Read the model definition and answer for the solid it produces. Units are mm, in the model's axes. Give positions to 0.01 mm unless a question says otherwise; leave off trailing zeros. Write each loop counter-clockwise with the first axis right and the second up, starting at its lowest first coordinate (ties: lowest second). Pieces come first, ordered by that corner, then holes. Notation, with made-up numbers: (-6, 25) -> (43, 25) arc R18 cw to (43, 37) -> close; hole circle Ø10 at (14, 70). An arc over 180 degrees is marked (long way). Use a Markdown table: item, result.
from build123d import *

# Parameters (mm, degrees)
SKETCH_1_R      = 1.65
EXTRUDE_1_DEPTH = 1.6


with BuildPart() as part:
    # 草图1 → 凸台-拉伸1 (new, symmetric)
    with BuildSketch(Plane.XY):
        Polygon((4.041451884, 0), (2.020725942, 3.5), (-2.020725942, 3.5), (-4.041451884, 0), (-2.020725942, -3.5), (2.020725942, -3.5), align=None)
        Circle(SKETCH_1_R, mode=Mode.SUBTRACT)
    extrude(amount=EXTRUDE_1_DEPTH, both=True)


solid = part.part
Item 1: For a pull along Y with two mould halves and no side action, classify faces 1 (the face through (3, -1.8, 0)), 2 (the face through (3.045, 1.726, 0.022)), 3 (the face through (-1.216, 1.115, -0.022)), 4 (the face through (2, 0, -1.6)) as +Y half, -Y half, draft (parallel to the pull), parting line (faces both ways), or undercut.
Return value:
| item | result |
|---|---|
| face 1 | -Y half |
| face 2 | +Y half |
| face 3 | undercut |
| face 4 | draft |
Item 2: Straight lines are drawn through the part: line 1 along Y through (x, z) = (0, -0.05); line 2 along X through (y, z) = (0.75, 1.35); line 3 along X through (y, z) = (-1.5, 1.25). For each, find the intervals that lie inside material, in ascending order. Write a range as [from, to].
Return value:
| item | result |
|---|---|
| line 1 | [-3.5, -1.65], [1.65, 3.5] |
| line 2 | [-3.61, -1.47], [1.47, 3.61] |
| line 3 | [-3.18, -0.69], [0.69, 3.18] |
Item 3: A cutting plane is placed at C-C (y = 1.5). Give the vertices of the cut face in (x, z), then the cut area to 3 significant figures.
Return value:
| item | result |
|---|---|
| outline | (-3.18, -1.6) -> (-0.69, -1.6) -> (-0.69, 1.6) -> (-3.18, 1.6) -> close; (0.69, -1.6) -> (3.18, -1.6) -> (3.18, 1.6) -> (0.69, 1.6) -> close |
| area | 15.9 mm^2 |
Item 4: A cutting plane is placed at B-B (z = -0.05). Give the vertices of the cut face in (x, y), then the cut area to 3 significant figures.
Return value:
| item | result |
|---|---|
| outline | (-4.04, 0) -> (-2.02, -3.5) -> (2.02, -3.5) -> (4.04, 0) -> (2.02, 3.5) -> (-2.02, 3.5) -> close; hole circle Ø3.3 at (0, 0) |
| area | 33.9 mm^2 |
Item 5: A cutting plane is placed at D-D (x = 3.25). Give the vertices of the cut face in (y, z).
Return value:
| item | result |
|---|---|
| outline | (-1.37, -1.6) -> (1.37, -1.6) -> (1.37, 1.6) -> (-1.37, 1.6) -> close |
Item 6: A cutting plane is placed at A-A (x = 0). Give the vertices of the cut face in (y, z).
Return value:
| item | result |
|---|---|
| outline | (-3.5, -1.6) -> (-1.65, -1.6) -> (-1.65, 1.6) -> (-3.5, 1.6) -> close; (1.65, -1.6) -> (3.5, -1.6) -> (3.5, 1.6) -> (1.65, 1.6) -> close |
